Design review of the part built by this model. Coordinates are the model's own, in mm. A direction names the side the tool comes from. Coordinates: 2 decimals unless noted, no trailing zeros. Loops run counter-clockwise (first coordinate to the right, second up) from the corner with the lowest first, then second, coordinate; pieces in that order, holes last. Notation, with made-up numbers: M -26.75,37 L 24.25,37 A25 cw 24.25,49 Z; hole C -36,21 d3. An arc over 180 degrees is marked long. Write item = value, one per line. Start each with the question number.
```python
from build123d import *

# Parameters (mm, degrees)
SKETCH1_W            = 60
SKETCH1_H            = 244
BOSS_EXTRUDE1_DEPTH  = 20
SKETCH2_W            = 15
SKETCH2_H            = 214
CUT_EXTRUDE1_DEPTH   = 128.21635115
M6_CLEARANCE_HOLE1_D = 6.6
CHAMFER1_SIZE        = 1


with BuildPart() as part:
    # Sketch1 → Boss-Extrude1 (new body)
    with BuildSketch(Plane.XY):
        Rectangle(SKETCH1_W, SKETCH1_H)
    extrude(amount=BOSS_EXTRUDE1_DEPTH)

    # Sketch2 → Cut-Extrude1 (cut, through all)
    with BuildSketch(Plane.XY.offset(20)):
        with Locations((-22.5, 0)):
            Rectangle(SKETCH2_W, SKETCH2_H)
        with Locations((22.5, 0)):
            Rectangle(SKETCH2_W, SKETCH2_H)
    extrude(amount=-CUT_EXTRUDE1_DEPTH, mode=Mode.SUBTRACT)

    # M6 Clearance Hole1 (through all)
    with Locations(Plane(origin=(0, 122, 0), x_dir=(1, 0, 0), z_dir=(0, 1, 0))):
        with Locations((-22.5, -10), (22.5, -10)):
            Hole(M6_CLEARANCE_HOLE1_D / 2)

    # Chamfer1
    chamfer1_edges = [part.edges().sort_by_distance(p)[0] for p in [
        (-30, 114.5, 20),
        (30, 114.5, 0),
        (-30, -114.5, 0),
        (30, 114.5, 20),
        (-30, -114.5, 20),
        (30, -114.5, 20),
        (-30, 114.5, 0),
        (30, -114.5, 0),
    ]]
    chamfer(chamfer1_edges, length=CHAMFER1_SIZE)


solid = part.part
```
(1) Tool access review of faces 1 (the flat face through (30, -115, 10)), 2 (the flat face through (15, -1, 10)), 3 (the flat face through (-26, -107, 10)): name each direction out of +Z, -Z, +X, -X, +Y, -Y from which nothing blocks a thin tool from reaching the whole face with its end or side.
(2) Mouldability with a two-part tool opening along Y and no side actions: class faces 4 (the flat face through (0, -122, 10)), 5 (the cylindrical face through (-25.55, -114.61, 11.26)), 6 (the flat face through (19, -107, 10)), 7 (the flat face through (0, 122, 10)) as +Y half, -Y half, draft (parallel to the pull), parting line (faces both ways), or undercut.
(3) Take a section at B-B (x = 22.5). State the section outline as (y, z) points, plus the area to 3 significant figures.
(4) Take a section at A-A (z = 10). State the section outline as (x, y) points.
(5) To check wall thickness, follow L1, parallel to X at y = -111, z = 10; L2, parallel to Z at x = 22.5, y = 114.25; L3, parallel to Y at x = 27.5, z = 13.5. State the ranges of each line that lie inside material, in increasing order.
(6) Insertion check: pin 1 (12 mm diameter, centred on y = -87.5, z = 15, fed in from -X); pin 2 (6 mm diameter, centred on y = 65, z = 3.5, fed in from +X). Each pin has a flat end and moves straight along its axis. Give the tip position at first contact, or say it passes through.
(7) Take a section at C-C (y = 102). State the section outline as (x, z) points.
Results list:
q1.face_1 = +Z, -Z, +X, +Y, -Y
q1.face_2 = +Z, -Z, +X
q1.face_3 = +Z, -Z, -X
q2.face_4 = -Y half
q2.face_5 = draft
q2.face_6 = undercut
q2.face_7 = +Y half
q3.outline = M -122,0 L -107,0 L -107,6.7 L -122,6.7 Z; M -122,13.3 L -107,13.3 L -107,20 L -122,20 Z; M 107,0 L 122,0 L 122,6.7 L 107,6.7 Z; M 107,13.3 L 122,13.3 L 122,20 L 107,20 Z
q3.area = 402 mm^2
q4.outline = M -30,-122 L -25.8,-122 L -25.8,-107 L -30,-107 Z; M -30,107 L -25.8,107 L -25.8,122 L -30,122 Z; M -19.2,-122 L 19.2,-122 L 19.2,-107 L 15,-107 L 15,107 L 19.2,107 L 19.2,122 L -19.2,122 L -19.2,107 L -15,107 L -15,-107 L -19.2,-107 Z; M 25.8,-122 L 30,-122 L 30,-107 L 25.8,-107 Z; M 25.8,107 L 30,107 L 30,122 L 25.8,122 Z
q5.L1 = -30 to -25.8, -19.2 to 19.2, 25.8 to 30
q5.L2 = 0 to 6.7, 13.3 to 20
q5.L3 = -122 to -107, 107 to 122
q6.pin_1 = -15
q6.pin_2 = 15
q7.outline = M -15,0 L 15,0 L 15,20 L -15,20 Z
